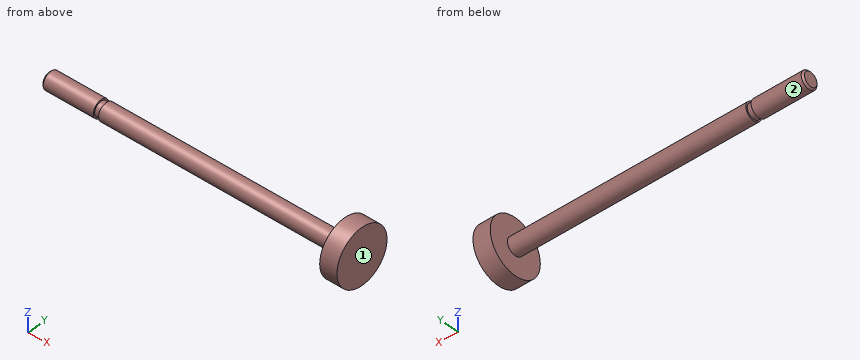
from build123d import *


with BuildPart() as part:
    # Sketch1 → Revolve1 (revolve)
    with BuildSketch(Plane.XY, mode=Mode.PRIVATE) as revolve1_sk:
        Polygon((0, 0), (0, 2.0095), (0.4905, 2.5), (15, 2.5), (15, 2.065), (16.5, 2.065), (16.5, 2.5), (85.5, 2.5), (85.5, 8), (90.5, 8), (90.5, 0), align=None)
    revolve(revolve1_sk.sketch.rotate(Axis((90.5, 0, 0), (-1, 0, 0)), 180), axis=Axis((90.5, 0, 0), (-1, 0, 0)))


solid = part.part
The listing builds one solid part. Answer for the finished solid, in the listing's coordinates (mm). Face numbers are marked on the shaded views. A direction names the side the tool comes from. Coordinates: 2 decimals unless noted, no trailing zeros. Write each loop counter-clockwise with the first axis right and the second up, starting at its lowest first coordinate (ties: lowest second). Pieces come first, ordered by that corner, then holes. Notation, with made-up numbers: M 86,30 L 145,30 A15 ccw 145,37 Z; hole C 39,58 d8. An arc over 180 degrees is marked long. Use one line per item in the form item = value.
Item 1: Find the intervals of material crossed by probe 1 along X at (y, z) = (1.75, 4); probe 2 along Z at (x, y) = (58.5, 0); probe 3 along Z at (x, y) = (9, 2.25), in increasing order.
Model answer:
probe_1 = 85.5 to 90.5
probe_2 = -2.5 to 2.5
probe_3 = -1.09 to 1.09
Item 2: Find section D-D, the plane z = 6. Give the vertices of the cut face in (x, y), plus the area to 3 significant figures.
Model answer:
outline = M 85.5,-5.29 L 90.5,-5.29 L 90.5,5.29 L 85.5,5.29 Z
area = 52.9 mm2
Item 3: Given P1, Ø5, axis at y = -3, z = -1.5, coming from the -X side; P2, Ø8, axis at x = 56, z = 6, coming from the -Y side; P3, Ø3, axis at x = 10, y = 2, coming from the -Z side, each flat-ended and moving along its own axis, determine where each tip first touches the part or whether it passes through.
Model answer:
P1 = 0
P2 = -1.5
P3 = -2.45
Item 4: Find section A-A, the plane z = 0. Give the vertices of the cut face in (x, y) (1 decimal), plus the area to 3 significant figures.
Model answer:
outline = M 0,-2 L 0.5,-2.5 L 15,-2.5 L 15,-2.1 L 16.5,-2.1 L 16.5,-2.5 L 85.5,-2.5 L 85.5,-8 L 90.5,-8 L 90.5,8 L 85.5,8 L 85.5,2.5 L 16.5,2.5 L 16.5,2.1 L 15,2.1 L 15,2.5 L 0.5,2.5 L 0,2 Z
area = 506 mm2
Item 5: Find section C-C, the plane x = 6. Give the vertices of the cut face in (y, z), plus the area to 3 significant figures.
Model answer:
outline = C 0,0 d5
area = 19.6 mm2
Item 6: For the marked faces 1 and 2, determine the directions among +Z, -Z, +X, -X, +Y, -Y from which every point of the face is accessible in a straight line to the end or side of a thin tool.
Model answer:
face_1 = +Z, -Z, +X, +Y, -Y
face_2 = -X
